The figure shows three views and two pictorial views of one solid part (mm, origin at its lowest corner). Answer the questions. A direction names the side the tool comes from. Coordinates: 2 decimals unless noted, no trailing zeros. Loops run counter-clockwise (first coordinate to the right, second up) from the corner with the lowest first, then second, coordinate; pieces in that order, holes last. Notation, with made-up numbers: M 87.5,17 L 118.5,17 A27 cw 118.5,33 Z; hole C 56,34.25 d6. An arc over 180 degrees is marked long. One line per item, written item: value. Start each with the question number.
1. Consider probe 1 along Z at (x, y) = (28, 13.5); probe 2 along Y at (x, z) = (50, 40.5); probe 3 along Z at (x, y) = (7, 55). Determine where each line is inside the solid, lowest interval first.
2. Determine the mould class of the marked faces 1, 2, 3 and 4 for opening direction Y: +Y half, -Y half, draft (parallel to the pull), parting line (faces both ways), or undercut.
3. Flat-ended cylindrical pins translate along their axes: pin 1 (8 mm diameter, centred on x = 60, y = 40, fed in from +Z); pin 2 (3 mm diameter, centred on x = 84.5, z = 34.5, fed in from -Y); pin 3 (3 mm diameter, centred on y = 72, z = 36.5, fed in from -X). Find the tip coordinate at first contact, or state that the pin passes through.
4. For the marked faces 5, 6, 7 and 8, determine the directions among +Z, -Z, +X, -X, +Y, -Y from which every point of the face is accessible in a straight line to the end or side of a thin tool.
5. The part is cut by section B-B (z = 34.5). Write down the section's boundary in (x, y).
6. The part is cut by section A-A (x = 50). Write down the section's boundary in (y, z), then the cut area to 3 significant figures.
7. The part is cut by section D-D (x = 83.5). Write down the section's boundary in (y, z), then the cut area to 3 significant figures.
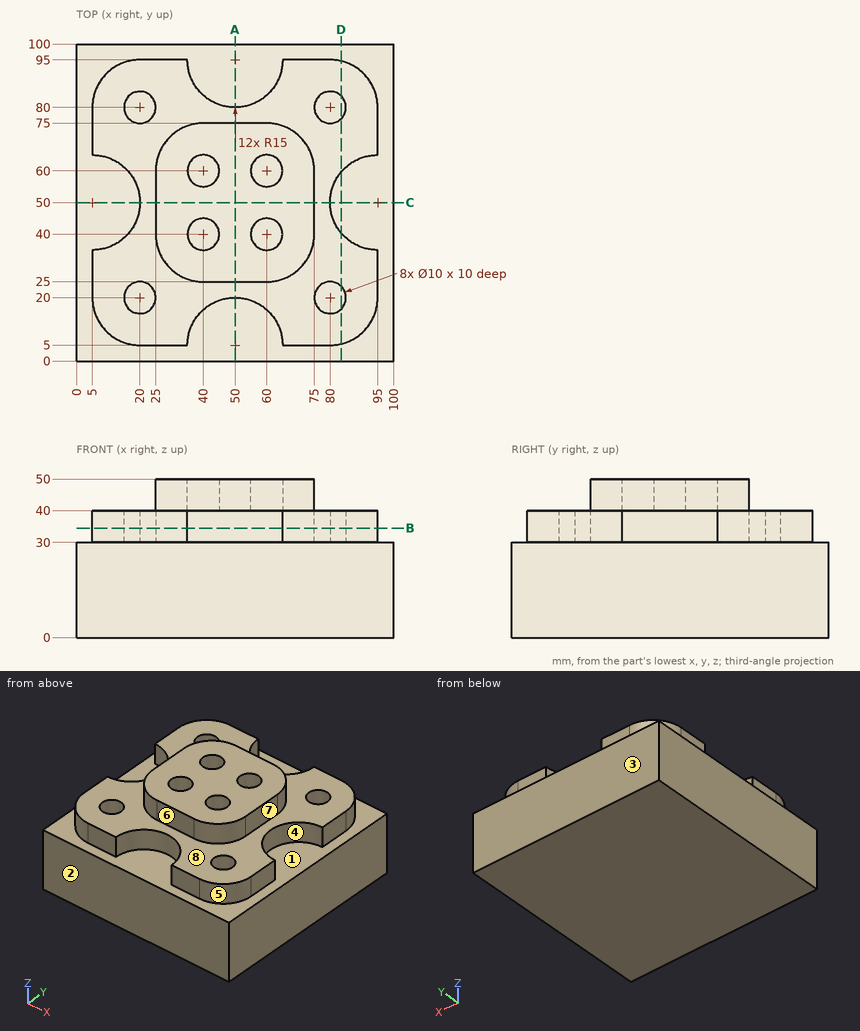
Answer block:
1. probe 1: z = 0 to 40
1. probe 2: y = 25 to 75
1. probe 3: z = 0 to 30
2. face 1: undercut
2. face 2: -Y half
2. face 3: +Y half
2. face 4: undercut
3. pin 1: stops at z = 40
3. pin 2: stops at y = 5.3
3. pin 3: stops at x = 5
4. face 5: +Z, +X, -Y
4. face 6: +Z, +X, -X, -Y
4. face 7: +Z, +X, +Y, -Y
4. face 8: +Z
5. outline: M 5,20 A15 ccw 20,5 L 35,5 A15 cw 65,5 L 80,5 A15 ccw 95,20 L 95,35 A15 cw 95,65 L 95,80 A15 ccw 80,95 L 65,95 A15 cw 35,95 L 20,95 A15 ccw 5,80 L 5,65 A15 cw 5,35 Z; hole C 20,20 d10; hole C 20,80 d10; hole C 80,20 d10; hole C 80,80 d10
6. outline: M 0,0 L 100,0 L 100,30 L 80,30 L 80,40 L 75,40 L 75,50 L 25,50 L 25,40 L 20,40 L 20,30 L 0,30 Z
6. area: 4,100 mm2
7. outline: M 0,0 L 100,0 L 100,30 L 94.59,30 L 94.59,40 L 83.57,40 L 83.57,30 L 76.43,30 L 76.43,40 L 59.63,40 L 59.63,30 L 40.37,30 L 40.37,40 L 23.57,40 L 23.57,30 L 16.43,30 L 16.43,40 L 5.41,40 L 5.41,30 L 0,30 Z
7. area: 3,560 mm2
